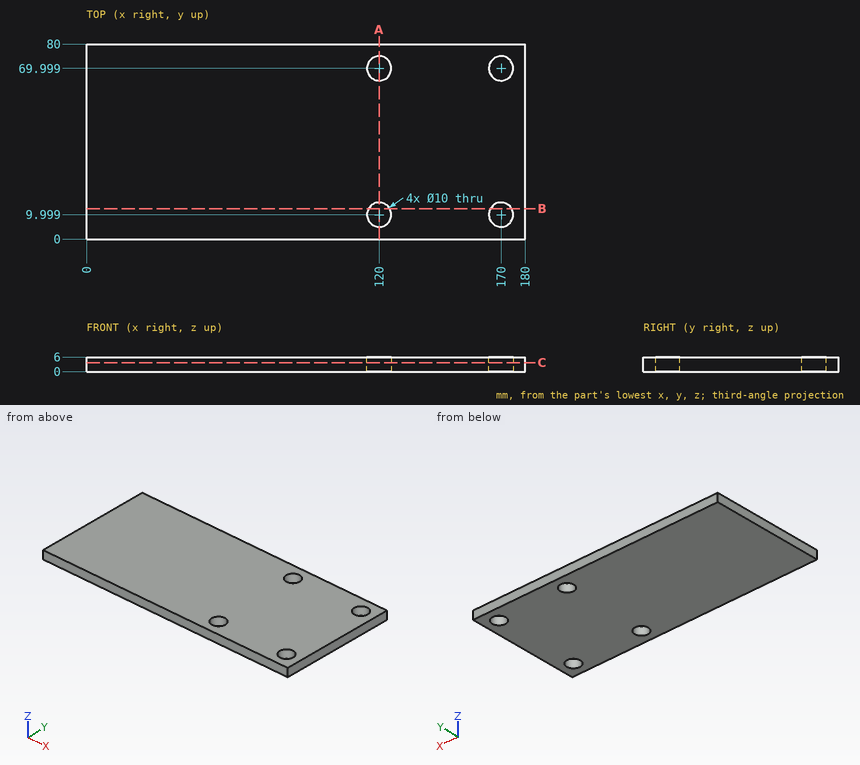
Source: three-view drawing plus pictorial views. Frame: mm from the lowest corner of the part. Give positions to 0.01 mm unless a question says otherwise; leave off trailing zeros. Order: outer loops, then holes, each group sorted by start corner. A loop starts at its lowest first (then second) coordinate and runs counter-clockwise, first axis right, second up. Notation, with made-up numbers: (12.25, -26) -> (71.25, -26) arc R32 ccw to (71.25, 6) -> close; hole circle Ø1 at (-15, 17). An arc over 180 degrees is marked (long way). Use a Markdown table: item, result.
Q1. Section C-C (z = 3.7). Return the cut outline in (x, y), and give its area (3 significant figures).
A:
| item | result |
|---|---|
| outline | (0, 0) -> (180, 0) -> (180, 80) -> (0, 80) -> close; hole circle Ø10 at (120, 10); hole circle Ø10 at (120, 70); hole circle Ø10 at (170, 10); hole circle Ø10 at (170, 70) |
| area | 14,100 mm^2 |
Q2. First-contact query: P1, Ø9, axis at x = 120, y = 70, coming from the +Z side. Flat tip, straight axial feed; report the tip coordinate or a pass-through.
A:
| item | result |
|---|---|
| P1 | through |
Q3. Section B-B (y = 12.5). Return the cut outline in (x, z), and give its area (3 significant figures).
A:
| item | result |
|---|---|
| outline | (0, 0) -> (115.67, 0) -> (115.67, 6) -> (0, 6) -> close; (124.33, 0) -> (165.67, 0) -> (165.67, 6) -> (124.33, 6) -> close; (174.33, 0) -> (180, 0) -> (180, 6) -> (174.33, 6) -> close |
| area | 976 mm^2 |
Q4. Material intervals for line 1 (Y direction, x = 120, z = 3.8); line 2 (X direction, y = 10.5, z = 2) (1 decimal); line 3 (X direction, y = 5.5, z = 4.4) (1 decimal), sorted ascending. Write a range as [from, to].
A:
| item | result |
|---|---|
| line 1 | [0, 5], [15, 65], [75, 80] |
| line 2 | [0, 115], [125, 165], [175, 180] |
| line 3 | [0, 117.8], [122.2, 167.8], [172.2, 180] |
Q5. Section A-A (x = 120). Return the cut outline in (y, z).
A:
| item | result |
|---|---|
| outline | (0, 0) -> (5, 0) -> (5, 6) -> (0, 6) -> close; (15, 0) -> (65, 0) -> (65, 6) -> (15, 6) -> close; (75, 0) -> (80, 0) -> (80, 6) -> (75, 6) -> close |
